For this review, take the finished solid that the model builds, in its own axes (mm). Coordinates: 2 decimals unless noted, no trailing zeros. Write each loop counter-clockwise with the first axis right and the second up, starting at its lowest first coordinate (ties: lowest second). Pieces come first, ordered by that corner, then holes. Notation, with made-up numbers: M -12,-20.5 L 46,-20.5 A13 cw 46,2.5 Z; hole C 34,50.25 d1. An arc over 180 degrees is marked long. Return JSON: item names as keys, results as strings.
```python
from build123d import *

# Parameters (mm, degrees)
SKETCH_1_W            = 280
SKETCH_1_H            = 260
EXTRUDE_1_DEPTH       = 15
CHAMFER_1_SIZE        = 5
HOLE_WIZARD_7_0_7_3_D = 7
HOLE_WIZARD_7_0_7_2_D = 7
HOLE_WIZARD_9_0_9_1_D = 9
HOLE_WIZARD_7_0_7_1_D = 7


with BuildPart() as part:
    # 草图1 → 凸台-拉伸1 (new body)
    with BuildSketch(Plane.XY):
        with Locations((140, -130)):
            Rectangle(SKETCH_1_W, SKETCH_1_H)
    extrude(amount=EXTRUDE_1_DEPTH)

    # 倒角1
    chamfer_1_edges = [part.edges().sort_by_distance(p)[0] for p in [
        (280, -260, 7.5),
        (0, -260, 7.5),
    ]]
    chamfer(chamfer_1_edges, length=CHAMFER_1_SIZE)

    # Ø7.0 (7) 直径孔3 (through all)
    with Locations(Plane(origin=(0, 0, 0), x_dir=(-1, 0, 0), z_dir=(0, 0, -1))):
        with Locations((-168, -185), (-112, -185), (-112, -251), (-168, -251)):
            Hole(HOLE_WIZARD_7_0_7_3_D / 2)

    # Ø7.0 (7) 直径孔2 (through all)
    with Locations(Plane.XY.offset(15)):
        with Locations((20, -6), (260, -6), (140, -6)):
            Hole(HOLE_WIZARD_7_0_7_2_D / 2)

    # Ø9.0 (9) 直径孔1 (through all)
    with Locations(Plane(origin=(0, 0, 0), x_dir=(-1, 0, 0), z_dir=(0, 0, -1))):
        with Locations((-268.5, -240.5), (-268.5, -195.5), (-211.5, -195.5), (-211.5, -240.5), (-68.5, -240.5), (-68.5, -195.5), (-11.5, -195.5), (-11.5, -240.5)):
            Hole(HOLE_WIZARD_9_0_9_1_D / 2)

    # Ø7.0 (7) 直径孔1 (through all)
    with Locations(Plane.XY.offset(15)):
        with Locations((6, -32), (274, -32), (274, -132), (6, -132)):
            Hole(HOLE_WIZARD_7_0_7_1_D / 2)


solid = part.part
```
1. Wall thickness on L1, parallel to Y at x = 168, z = 8.75; L2, parallel to Y at x = 268.5, z = 8; L3, parallel to Y at x = 260, z = 6.75: over which ranges is each line inside the solid? List them lowest first. Write a range as from..to.
Checks:
{"L1": "-260..-254.5, -247.5..-188.5, -181.5..0", "L2": "-260..-245, -236..-200, -191..0", "L3": "-260..-9.5, -2.5..0"}
2. We need section B-B (y = -32). State the section outline as (x, z) points.
Checks:
{"outline": "M 0,0 L 2.5,0 L 2.5,15 L 0,15 Z; M 9.5,0 L 270.5,0 L 270.5,15 L 9.5,15 Z; M 277.5,0 L 280,0 L 280,15 L 277.5,15 Z"}
3. We need section A-A (x = 140). State the section outline as (y, z) points, plus the area to 4 significant figures.
Checks:
{"outline": "M -260,0 L -9.5,0 L -9.5,15 L -260,15 Z; M -2.5,0 L 0,0 L 0,15 L -2.5,15 Z", "area": "3,795 mm2"}
4. We need section C-C (x = 112). State the section outline as (y, z) points, plus the area to 3 significant figures.
Checks:
{"outline": "M -260,0 L -254.5,0 L -254.5,15 L -260,15 Z; M -247.5,0 L -188.5,0 L -188.5,15 L -247.5,15 Z; M -181.5,0 L 0,0 L 0,15 L -181.5,15 Z", "area": "3,690 mm2"}
5. Draft analysis for pull direction X (two halves, no side actions). For faces 1 (the face through (115.233, -252.341, 7.605)), 2 (the face through (171.34, -183.95, 7.61)), 3 (the face through (138, -128, 0)), state which applies: +X half, -X half, draft (parallel to the pull), parting line (faces both ways), or undercut.
Checks:
{"face 1": "undercut", "face 2": "undercut", "face 3": "draft"}
